Verification items for this drawing (mm, ordinates from the low corner). A direction names the side the tool comes from. Round coordinates to 2 decimals unless told otherwise and drop trailing zeros. Loops run counter-clockwise (first coordinate to the right, second up) from the corner with the lowest first, then second, coordinate; pieces in that order, holes last. Notation, with made-up numbers: (35.5, 56.25) -> (72.5, 56.25) arc R24 cw to (72.5, 86.25) -> close; hole circle Ø6 at (-22, 59.25). An arc over 180 degrees is marked (long way). Use a Markdown table: item, result. Add a question column.
Q1. Sectioned sample at A-A, the plane z = 12.5. Enter the section's corners in (x, y).
Q2. Release check for a two-part mould opening along Z. For the marked faces 1, 2, 3 and 4 record: released by +Z, released by -Z, zero draft, split by the parting line, or undercut.
Q3. Sectioned sample at B-B, the plane x = 10. Enter the section's corners in (y, z), then the cut area to 3 significant figures.
Q4. Set-up check for the marked faces 5 and 6: record each of +Z, -Z, +X, -X, +Y, -Y from which the full face is reachable in a straight line by a thin tool's end or side.
Q5. Sectioned sample at C-C, the plane y = 9.25. Enter the section's corners in (x, z), then the cut area to 3 significant figures.
Q6. Material ranges on L1, parallel to X at y = 0.5, z = 27.5; L2, parallel to Z at x = 8.5, y = 3 (3 decimals), recorded low to high.
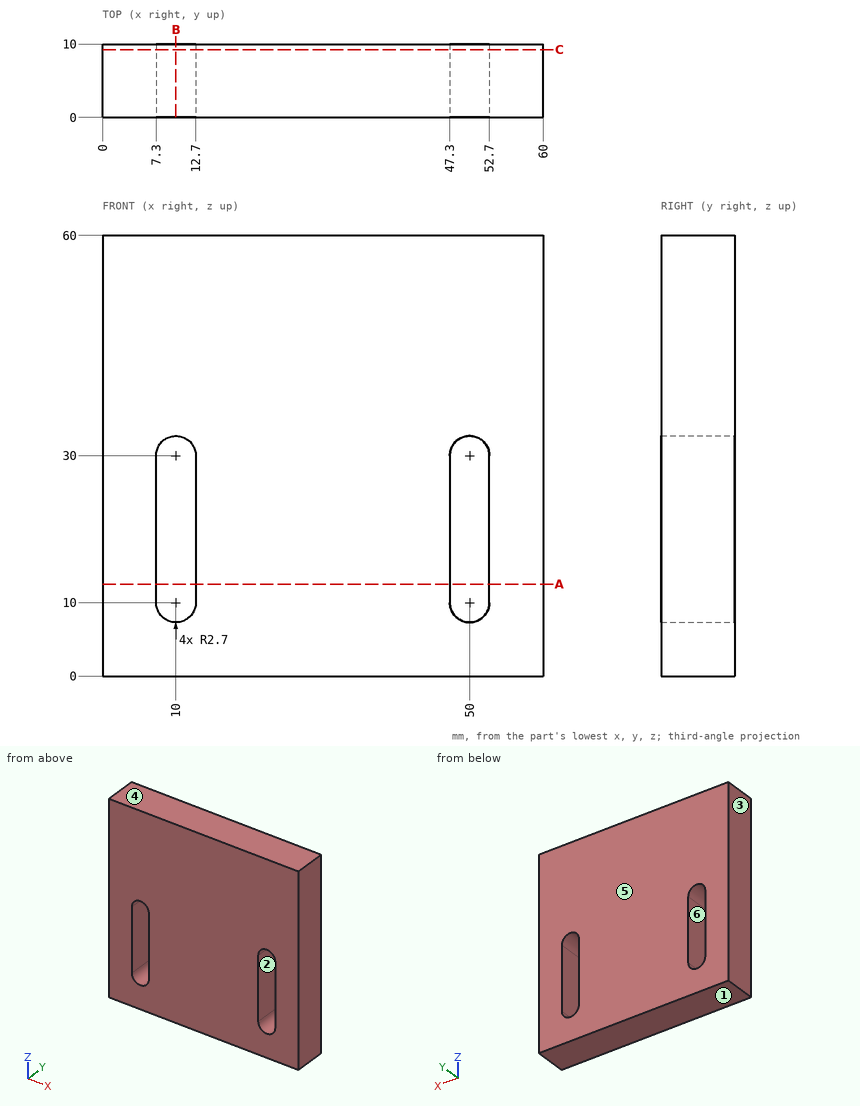
Values:
| question | item | result |
|---|---|---|
| 1 | outline | (0, 0) -> (7.3, 0) -> (7.3, 10) -> (0, 10) -> close; (12.7, 0) -> (47.3, 0) -> (47.3, 10) -> (12.7, 10) -> close; (52.7, 0) -> (60, 0) -> (60, 10) -> (52.7, 10) -> close |
| 2 | face 1 | released by -Z |
| 2 | face 2 | undercut |
| 2 | face 3 | zero draft |
| 2 | face 4 | released by +Z |
| 3 | outline | (0, 0) -> (10, 0) -> (10, 7.3) -> (0, 7.3) -> close; (0, 32.7) -> (10, 32.7) -> (10, 60) -> (0, 60) -> close |
| 3 | area | 346 mm^2 |
| 4 | face 5 | +Z, -Z, +X, -X, +Y |
| 4 | face 6 | +Y, -Y |
| 5 | outline | (0, 0) -> (60, 0) -> (60, 60) -> (0, 60) -> close; hole (7.3, 10) arc R2.7 ccw to (12.7, 10) -> (12.7, 30) arc R2.7 ccw to (7.3, 30) -> close; hole (47.3, 10) arc R2.7 ccw to (52.7, 10) -> (52.7, 30) arc R2.7 ccw to (47.3, 30) -> close |
| 5 | area | 3,340 mm^2 |
| 6 | L1 | 0 to 7.3, 12.7 to 47.3, 52.7 to 60 |
| 6 | L2 | 0 to 7.755, 32.245 to 60 |
